Input: dimensioned drawing with shaded views. Units: mm. Origin: part minimum x, y, z. Coordinates: 2 decimals unless noted, no trailing zeros. Write each loop counter-clockwise with the first axis right and the second up, starting at its lowest first coordinate (ties: lowest second). Pieces come first, ordered by that corner, then holes. Notation, with made-up numbers: M -0.5,57.25 L 21.5,57.25 A22 ccw 21.5,63.25 Z; hole C -13.5,57.5 d11. An arc over 180 degrees is marked long. Use one line per item in the form item = value.
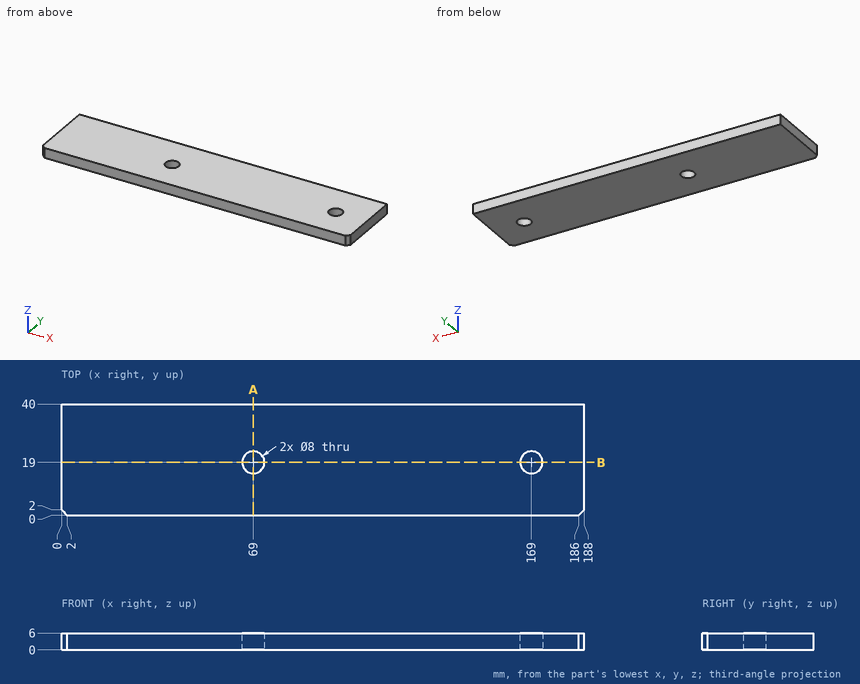
(1) Line query: probe 1 along Y at (x, z) = (169, 2.75); probe 2 along X at (y, z) = (21, 3.85); probe 3 along X at (y, z) = (15.5, 5.5). Output: solid intervals per line, ascending.
Computed:
probe_1 = 0 to 15, 23 to 40
probe_2 = 0 to 65.54, 72.46 to 165.54, 172.46 to 188
probe_3 = 0 to 67.06, 70.94 to 167.06, 170.94 to 188
(2) Section query B-B on y = 19. Return the cut outline in (x, z).
Computed:
outline = M 0,0 L 65,0 L 65,6 L 0,6 Z; M 73,0 L 165,0 L 165,6 L 73,6 Z; M 173,0 L 188,0 L 188,6 L 173,6 Z
(3) Section query A-A on x = 69. Return the cut outline in (y, z).
Computed:
outline = M 0,0 L 15,0 L 15,6 L 0,6 Z; M 23,0 L 40,0 L 40,6 L 23,6 Z
